```python
from build123d import *

# Parameters (mm, degrees)
SKETCH_1_W             = 120
SKETCH_1_H             = 10
EXTRUDE_1_DEPTH        = 20
SKETCH_2_R             = 1.09
CUT_EXTRUDE_1_DEPTH    = 3
SKETCH_4_R             = 0.825
CUT_EXTRUDE_2_DEPTH    = 30
PATTERN_LINEAR_1_COUNT = 10
PATTERN_LINEAR_1_PITCH = 12
CHAMFER_1_SIZE         = 2
MM_1_D                 = 5
MM_1_DEPTH             = 15
MM_1_TIP               = 1.502151548
HOLE_WIZARD_M5_1_D     = 5.5
HOLE_WIZARD_M5_1_DEPTH = 15
HOLE_WIZARD_M5_1_TIP   = 1.652366702


with BuildPart() as part:
    # 草图1 → 凸台-拉伸1 (new body)
    with BuildSketch(Plane(origin=(0, 0, 0), x_dir=(1, 0, 0), z_dir=(0, 1, 0))):
        Rectangle(SKETCH_1_W, SKETCH_1_H)
    extrude(amount=EXTRUDE_1_DEPTH)

    # 草图2 → 切除-拉伸1 (cut)
    with BuildSketch(Plane(origin=(0, 20, 0), x_dir=(1, 0, 0), z_dir=(0, 1, 0))):
        with Locations(Location((-54, 0, 0), (0, 0, 270))):
            Circle(SKETCH_2_R)
    cut_extrude_1 = extrude(amount=-CUT_EXTRUDE_1_DEPTH, mode=Mode.SUBTRACT)

    # 草图4 → 切除-拉伸2 (cut)
    with BuildSketch(Plane(origin=(0, 17, 0), x_dir=(1, 0, 0), z_dir=(0, 1, 0))):
        with Locations(Location((-54, 0, 0), (0, 0, 270))):
            Circle(SKETCH_4_R)
    cut_extrude_2 = extrude(amount=-CUT_EXTRUDE_2_DEPTH, mode=Mode.SUBTRACT)

    # 阵列(线性)1: 切除-拉伸1, 切除-拉伸2 ×10
    with Locations(*[(i * PATTERN_LINEAR_1_PITCH, 0, 0) for i in range(1, PATTERN_LINEAR_1_COUNT)]):
        add(cut_extrude_1, mode=Mode.SUBTRACT)
        add(cut_extrude_2, mode=Mode.SUBTRACT)

    # 倒角1
    chamfer_1_edges = [part.edges().sort_by_distance(p)[0] for p in [
        (-60, 20, 0),
        (60, 20, 0),
        (-60, 0, 0),
        (60, 0, 0),
    ]]
    chamfer(chamfer_1_edges, length=CHAMFER_1_SIZE)

    # 大小mm 暗销孔1
    with Locations(Plane.XY.offset(5)):
        with Locations((36, 10), (-36, 10)):
            Hole(MM_1_D / 2, depth=MM_1_DEPTH)
            with Locations((0, 0, -(MM_1_DEPTH + MM_1_TIP / 2))):  # 118° drill point
                Cone(0, MM_1_D / 2, MM_1_TIP, mode=Mode.SUBTRACT)

    # M5 间隙孔1
    with Locations(Plane.XY.offset(5)):
        with Locations((0, 10)):
            Hole(HOLE_WIZARD_M5_1_D / 2, depth=HOLE_WIZARD_M5_1_DEPTH)
            with Locations((0, 0, -(HOLE_WIZARD_M5_1_DEPTH + HOLE_WIZARD_M5_1_TIP / 2))):  # 118° drill point
                Cone(0, HOLE_WIZARD_M5_1_D / 2, HOLE_WIZARD_M5_1_TIP, mode=Mode.SUBTRACT)


solid = part.part
```
Here's how the part is built. I have some questions about the finished solid (model axes, mm). A direction names the side the tool comes from. Round coordinates to 2 decimals unless told otherwise and drop trailing zeros. Order: outer loops, then holes, each group sorted by start corner. A loop starts at its lowest first (then second) coordinate and runs counter-clockwise, first axis right, second up. Notation, with made-up numbers: M 67,31.25 L 71,31.25 A19 ccw 71,59.25 Z; hole C 27.25,0.25 d9. An arc over 180 degrees is marked long. Answer as CSV lines item,"result".
Item 1: Please list where these lines run through material, in increasing order: L1, parallel to X at y = 9.75, z = 1; L2, parallel to Y at x = 0, z = -1.25; L3, parallel to Z at x = 42, y = 13 (3 decimals). Write a range as [from, to].
From the geometry:
L1,"[-60, -38.49], [-33.51, -2.74], [2.74, 33.51], [38.49, 60]"
L2,"[0, 7.25], [12.75, 20]"
L3,"[-5, -0.825], [0.825, 5]"
Item 2: Imagine slicing it at B-B on y = 3.5. Give the number of separate pieces and of enclosed holes in the cut face, and give its area (3 significant figures).
From the geometry:
separate pieces,"1"
enclosed holes,"10"
area,"1,180 mm2"
Item 3: We'd pull the mould along Z, two halves only. Please class faces 1 (the cylindrical face through (31.08, 18.52, -0.14)), 2 (the flat face through (-1, 5, 5)), 3 (the flat face through (59, 19, 0)): +Z half, -Z half, draft (parallel to the pull), parting line (faces both ways), or undercut.
From the geometry:
face 1,"undercut"
face 2,"+Z half"
face 3,"draft"
Item 4: Imagine slicing it at C-C on x = -36. List the corners of the cut face in (y, z) for me, and give its area (3 significant figures).
From the geometry:
outline,"M 0,-5 L 7.5,-5 L 7.5,5 L 0,5 Z; M 12.5,-5 L 20,-5 L 20,5 L 12.5,5 Z"
area,"150 mm2"
Item 5: For pin 1 (2.5 mm diameter, centred on x = -18, z = 0, fed in from -Y); pin 2 (1.1 mm diameter, centred on x = 42, z = 0.5, fed in from +Y), each with a flat end and sliding along its axis, tell me the tip position at first contact or that it passes through.
From the geometry:
pin 1,"y = 0"
pin 2,"y = 17"
Item 6: Imagine slicing it at A-A on x = 0. List the corners of the cut face in (y, z) for me.
From the geometry:
outline,"M 0,-5 L 7.25,-5 L 7.25,5 L 0,5 Z; M 12.75,-5 L 20,-5 L 20,5 L 12.75,5 Z"
Item 7: Which directions (+Z, -Z, +X, -X, +Y, -Y) give clear straight access to the entire face, cutting with the end or side of a thin tool? Please do faces 4 (the cylindrical face through (-40.92, 18.52, -0.14)), 5 (the flat face through (-59, 19, 0)).
From the geometry:
face 4,"+Y"
face 5,"+Z, -Z, -X, +Y"
